Geometry check sheet. Reference: the model listing, model coordinates, mm. A direction names the side the tool comes from. Coordinates: 2 decimals unless noted, no trailing zeros. Write each loop counter-clockwise with the first axis right and the second up, starting at its lowest first coordinate (ties: lowest second). Pieces come first, ordered by that corner, then holes. Notation, with made-up numbers: (-16.75, 39.5) -> (12.25, 39.5) arc R20 cw to (12.25, 72.5) -> close; hole circle Ø8 at (9.25, 67.5). An arc over 180 degrees is marked (long way). Answer in a Markdown table with one row per item. Add a question column.
Q1. Tool access check on faces 5 (the face through (10, -3, 135)), 6 (the face through (12, -1.4, 103)), 7 (the face through (10, 1, -147.5)), 8 (the face through (3, 4, 5.05)), 9 (the face through (16, -2, 0)). Record the directions out of +Z, -Z, +X, -X, +Y, -Y that give a thin tool (end or side, any length) a straight path to the whole face; none if there is none.
Q2. Thickness scan on line 1 (Z direction, x = 14, y = 4); line 2 (X direction, y = 1.35, z = -81); line 3 (Z direction, x = 14, y = 1.2). Record the ranges inside material, lowest first.
Q3. Gauge pin test, flat ends, axial feed: P1, Ø5, axis at x = 14, z = -101, coming from the +Y side; P2, Ø4, axis at x = 15.5, z = -81.5, coming from the -Y side; P3, Ø2.5, axis at x = 8, y = -4.5, coming from the -Z side; P4, Ø5, axis at x = 8, z = 1.5, coming from the -Y side. Record the tip position at first contact, or that the pin passes through.
Q4. Section check B-B, the plane z = 0. Record the boundary of the cut face in (x, y).
Q5. Section check A-A, the plane z = -89. Record the boundary of the cut face in (x, y), and give its area (3 significant figures).
Q6. Release check for a two-part mould opening along X. For faces 1 (the face through (14.867, -3.732, -77.095)), 2 (the face through (13.512, 0.831, -98.804)), 3 (the face through (11.05, 3.52, 0.11)), 4 (the face through (10, 1, 147.5)) record: pulls with the +X half, pulls with the -X half, needs draft (parallel to the pull), parting line crosses it, or undercut.
```python
from build123d import *

# Parameters (mm, degrees)
SKETCH1_W                                            = 295
SKETCH1_H                                            = 12
BOSS_EXTRUDE1_DEPTH                                  = 20
CUT_EXTRUDE1_DEPTH                                   = 150.33268229
CUT_EXTRUDE2_DEPTH                                   = 7.1
SKETCH4_W                                            = 20
SKETCH4_H                                            = 25
CUT_EXTRUDE3_DEPTH                                   = 3
SKETCH5_W                                            = 10
SKETCH5_H                                            = 35.2
CUT_EXTRUDE4_DEPTH                                   = 3
SKETCH7_R                                            = 1.5
CUT_EXTRUDE6_DEPTH                                   = 3
M4_TAPPED_HOLE2_D                                    = 3.3
M4_TAPPED_HOLE2_DEPTH                                = 10.1
M4_TAPPED_HOLE2_TIP                                  = 0.991420021
M4_TAPPED_HOLE1_D                                    = 3.3
M4_TAPPED_HOLE1_DEPTH                                = 10.1
M4_TAPPED_HOLE1_TIP                                  = 0.991420021
CBORE_FOR_M4_HEXAGON_SOCKET_HEAD_CAP_SCR_D           = 4.5
CBORE_FOR_M4_HEXAGON_SOCKET_HEAD_CAP_SCR_CBORE_D     = 8
CBORE_FOR_M4_HEXAGON_SOCKET_HEAD_CAP_SCR_CBORE_DEPTH = 4.6
CHAMFER1_SIZE                                        = 2


with BuildPart() as part:
    # Sketch1 → Boss-Extrude1 (new body)
    with BuildSketch(Plane(origin=(0, 0, 0), x_dir=(0, 0, -1), z_dir=(1, 0, 0))):
        Rectangle(SKETCH1_W, SKETCH1_H)
    extrude(amount=BOSS_EXTRUDE1_DEPTH)

    # Sketch2 → Cut-Extrude1 (cut, through all)
    with BuildSketch(Plane.XZ.offset(6)):
        with BuildLine():
            Line((0, 5.05), (6, 5.05))
            ThreePointArc((6, 5.05), (11.05, 0), (6, -5.05))
            Line((6, -5.05), (0, -5.05))
            ThreePointArc((0, -5.05), (-5.05, 0), (0, 5.05))
        make_face()
    extrude(amount=-CUT_EXTRUDE1_DEPTH, mode=Mode.SUBTRACT)

    # Sketch3 → Cut-Extrude2 (cut)
    with BuildSketch(Plane.XZ.offset(6)):
        with BuildLine():
            Line((0, 10), (6, 10))
            ThreePointArc((6, 10), (16, 0), (6, -10))
            Line((6, -10), (0, -10))
            ThreePointArc((0, -10), (-10, 0), (0, 10))
        make_face()
    extrude(amount=-CUT_EXTRUDE2_DEPTH, mode=Mode.SUBTRACT)

    # Sketch4 → Cut-Extrude3 (cut)
    with BuildSketch(Plane(origin=(0, -6, 0), x_dir=(1, 0, 0), z_dir=(0, 1, 0))):
        with Locations((10, -135)):
            Rectangle(SKETCH4_W, SKETCH4_H)
        with Locations((10, 135)):
            Rectangle(SKETCH4_W, SKETCH4_H)
    extrude(amount=CUT_EXTRUDE3_DEPTH, mode=Mode.SUBTRACT)

    # Sketch5 → Cut-Extrude4 (cut)
    with BuildSketch(Plane(origin=(0, 6, 0), x_dir=(1, 0, 0), z_dir=(0, 1, 0))):
        with Locations((15, 91)):
            Rectangle(SKETCH5_W, SKETCH5_H)
        with Locations((15, -91)):
            Rectangle(SKETCH5_W, SKETCH5_H)
    extrude(amount=-CUT_EXTRUDE4_DEPTH, mode=Mode.SUBTRACT)

    # Sketch7 → Cut-Extrude6 (cut)
    with BuildSketch(Plane(origin=(0, 6, 0), x_dir=(1, 0, 0), z_dir=(0, 1, 0))):
        with Locations((10, 108.6)):
            Circle(SKETCH7_R)
        with Locations((10, 73.4)):
            Circle(SKETCH7_R)
        with Locations((10, -73.4)):
            Circle(SKETCH7_R)
        with Locations((10, -108.6)):
            Circle(SKETCH7_R)
    extrude(amount=-CUT_EXTRUDE6_DEPTH, mode=Mode.SUBTRACT)

    # M4 Tapped Hole2
    with Locations(Plane(origin=(0, -3, 0), x_dir=(-1, 0, 0), z_dir=(0, -1, 0))):
        with Locations((-10, -141), (-10, -129)):
            Hole(M4_TAPPED_HOLE2_D / 2, depth=M4_TAPPED_HOLE2_DEPTH)
            with Locations((0, 0, -(M4_TAPPED_HOLE2_DEPTH + M4_TAPPED_HOLE2_TIP / 2))):  # 118° drill point
                Cone(0, M4_TAPPED_HOLE2_D / 2, M4_TAPPED_HOLE2_TIP, mode=Mode.SUBTRACT)

    # M4 Tapped Hole1
    with Locations(Plane(origin=(0, -3, 0), x_dir=(-1, 0, 0), z_dir=(0, -1, 0))):
        with Locations((-10, 141), (-10, 129)):
            Hole(M4_TAPPED_HOLE1_D / 2, depth=M4_TAPPED_HOLE1_DEPTH)
            with Locations((0, 0, -(M4_TAPPED_HOLE1_DEPTH + M4_TAPPED_HOLE1_TIP / 2))):  # 118° drill point
                Cone(0, M4_TAPPED_HOLE1_D / 2, M4_TAPPED_HOLE1_TIP, mode=Mode.SUBTRACT)

    # CBORE for M4 Hexagon socket head cap screws1 (through all)
    with Locations(Plane(origin=(0, -6, 0), x_dir=(-1, 0, 0), z_dir=(0, -1, 0))):
        with Locations((-14, 101), (-14, 81), (-14, -81), (-14, -101)):
            CounterBoreHole(CBORE_FOR_M4_HEXAGON_SOCKET_HEAD_CAP_SCR_D / 2, CBORE_FOR_M4_HEXAGON_SOCKET_HEAD_CAP_SCR_CBORE_D / 2, CBORE_FOR_M4_HEXAGON_SOCKET_HEAD_CAP_SCR_CBORE_DEPTH)

    # Chamfer1
    chamfer1_edges = [part.edges().sort_by_distance(p)[0] for p in [
        (20, 1.5, 147.5),
        (0, 1.5, 147.5),
        (0, 1.5, -147.5),
        (20, 1.5, -147.5),
    ]]
    chamfer(chamfer1_edges, length=CHAMFER1_SIZE)


solid = part.part
```
Calculated:
| question | item | result |
|---|---|---|
| 1 | face 5 | +Z, +X, -X, -Y |
| 1 | face 6 | -Y |
| 1 | face 7 | -Z, +X, -X, +Y, -Y |
| 1 | face 8 | -X, +Y, -Y |
| 1 | face 9 | -X, -Y |
| 2 | line 1 | z = -147.5 to -108.6, -73.4 to 73.4, 108.6 to 147.5 |
| 2 | line 2 | x = 0 to 11.75, 16.25 to 20 |
| 2 | line 3 | z = -147.5 to -103.25, -98.75 to -83.25, -78.75 to 78.75, 83.25 to 98.75, 103.25 to 147.5 |
| 3 | P1 | stops at y = 3 |
| 3 | P2 | stops at y = -1.4 |
| 3 | P3 | stops at z = -122.5 |
| 3 | P4 | passes through |
| 4 | outline | (11.05, 1.1) -> (16, 1.1) -> (16, -6) -> (20, -6) -> (20, 6) -> (11.05, 6) -> close |
| 5 | outline | (0, -6) -> (20, -6) -> (20, 3) -> (10, 3) -> (10, 6) -> (0, 6) -> close |
| 5 | area | 210 mm² |
| 6 | face 1 | undercut |
| 6 | face 2 | undercut |
| 6 | face 3 | pulls with the -X half |
| 6 | face 4 | needs draft |
